CAD build for the part. Positions are in the model's coordinates, mm. Round coordinates to 2 decimals unless told otherwise and drop trailing zeros. Order: outer loops, then holes, each group sorted by start corner. A loop starts at its lowest first (then second) coordinate and runs counter-clockwise, first axis right, second up. Notation, with made-up numbers: M 12.5,17 L 41.5,17 A30 cw 41.5,53 Z; hole C 77,18 d5. An arc over 180 degrees is marked long. Answer as a JSON object with one key per item and string values. Group by question number.
```python
from build123d import *

# Parameters (mm, degrees)
EXTRUDE_1_DEPTH     = 15
SKETCH_2_R          = 17.5
CUT_EXTRUDE_1_DEPTH = 155.878985017
SKETCH_3_R          = 17.5
CUT_EXTRUDE_2_DEPTH = 155.878985017


with BuildPart() as part:
    # 草图1 → 凸台-拉伸1 (new body)
    with BuildSketch(Plane(origin=(0, 0, 0), x_dir=(0, 0, -1), z_dir=(1, 0, 0))):
        with BuildLine():
            Line((22.5, 0), (22.5, -130))
            ThreePointArc((22.5, -130), (0, -152.5), (-22.5, -130))
            Line((-22.5, -130), (-22.5, 0))
            ThreePointArc((-22.5, 0), (0, 22.5), (22.5, 0))
        make_face()
    extrude(amount=EXTRUDE_1_DEPTH)

    # 草图2 → 切除-拉伸1 (cut, through all)
    with BuildSketch(Plane(origin=(15, 0, 0), x_dir=(0, 0, -1), z_dir=(1, 0, 0))):
        Circle(SKETCH_2_R)
    extrude(amount=-CUT_EXTRUDE_1_DEPTH, mode=Mode.SUBTRACT)

    # 草图3 → 切除-拉伸2 (cut, through all)
    with BuildSketch(Plane.ZY):
        with Locations((0, -130)):
            Circle(SKETCH_3_R)
    extrude(amount=-CUT_EXTRUDE_2_DEPTH, mode=Mode.SUBTRACT)


solid = part.part
```
Item 1: Cut at D-D, the plane z = 14.5. Give the cut face in (x, y), and give its area (3 significant figures).
Item 2: Cut at A-A, the plane z = 0. Give the cut face in (x, y).
Item 3: Two-plate mould, pull along Z, no slides. Class faces 1 (the face through (7.395, 22.495, 0.495)), 2 (the face through (7, -64, -22.5)), 3 (the face through (7.4, -112.65, -2.28)): +Z half, -Z half, draft (parallel to the pull), parting line (faces both ways), or undercut.
Item 4: Flat gauge pins, fed straight in: pin 1 Ø2 at (x, z) = (2.5, 9) entering from +Y; pin 2 Ø21 at (y, z) = (0, 0) entering from -X; pin 3 Ø8 at (x, z) = (3, 17.5) entering from +Y; pin 4 Ø6 at (x, z) = (6.5, -2.5) entering from -Y. Where does each tip first touch, or does it go through?
Item 5: Drill centre lines: line 1 (Y direction, x = 7, z = 0); line 2 (Y direction, x = 6.75, z = -12.5); line 3 (Z direction, x = 5.75, y = -120). Where is each one in solid material? Low to high. Write a range as [from, to].
Item 6: Cut at C-C, the plane y = -125.5. Give the cut face in (x, z).
Item 7: Cut at B-B, the plane x = 1.5. Give the cut face in (y, z), and give its area (3 significant figures).
Response values:
{
 "1": {"outline": "M 0,-147.2 L 15,-147.2 L 15,-139.8 L 0,-139.8 Z; M 0,-120.2 L 15,-120.2 L 15,-9.8 L 0,-9.8 Z; M 0,9.8 L 15,9.8 L 15,17.2 L 0,17.2 Z", "area": "1,880 mm^2"},
 "2": {"outline": "M 0,-152.5 L 15,-152.5 L 15,-147.5 L 0,-147.5 Z; M 0,-112.5 L 15,-112.5 L 15,-17.5 L 0,-17.5 Z; M 0,17.5 L 15,17.5 L 15,22.5 L 0,22.5 Z"},
 "3": {"face 1": "parting line", "face 2": "-Z half", "face 3": "undercut"},
 "4": {"pin 1": "y = 21.03", "pin 2": "through", "pin 3": "y = 18", "pin 4": "y = -152.5"},
 "5": {"line 1": "[-152.5, -147.5], [-112.5, -17.5], [17.5, 22.5]", "line 2": "[-148.71, -142.25], [-117.75, -12.25], [12.25, 18.71]", "line 3": "[-22.5, -14.36], [14.36, 22.5]"},
 "6": {"outline": "M 0,-22.5 L 15,-22.5 L 15,-16.91 L 0,-16.91 Z; M 0,16.91 L 15,16.91 L 15,22.5 L 0,22.5 Z"},
 "7": {"outline": "M -130,-22.5 L 0,-22.5 A22.5 ccw 0,22.5 L -130,22.5 A22.5 ccw Z; hole C -130,0 d35; hole C 0,0 d35", "area": "5,520 mm^2"}
}
